Geometry: final body of the model. Coordinates: model frame, mm. Round coordinates to 2 decimals unless told otherwise and drop trailing zeros. Loops run counter-clockwise (first coordinate to the right, second up) from the corner with the lowest first, then second, coordinate; pieces in that order, holes last. Notation, with made-up numbers: M 9.25,-30.75 L 24.25,-30.75 A27 ccw 24.25,0.25 Z; hole C 74.25,1.5 d6. An arc over 180 degrees is marked long. Answer as a JSON object with one key per item and string values.
```python
from build123d import *

# Parameters (mm, degrees)
SKETCH1_R           = 2
SKETCH1_R_2         = 3
BOSS_EXTRUDE1_DEPTH = 5
SKETCH2_R           = 2
CUT_EXTRUDE1_DEPTH  = 36.174564674


with BuildPart() as part:
    # Sketch1 → Boss-Extrude1 (new body)
    with BuildSketch(Plane.XY):
        with BuildLine():
            Line((-3.972684511, 30.466666667), (-7.448783458, 0.875))
            ThreePointArc((-7.448783458, 0.875), (0, -7.5), (7.448783458, 0.875))
            Line((7.448783458, 0.875), (3.972684511, 30.466666667))
            ThreePointArc((3.972684511, 30.466666667), (0, 34), (-3.972684511, 30.466666667))
        make_face()
        with Locations((0, 30)):
            Circle(SKETCH1_R, mode=Mode.SUBTRACT)
        Circle(SKETCH1_R_2, mode=Mode.SUBTRACT)
    extrude(amount=BOSS_EXTRUDE1_DEPTH)

    # Sketch2 → Cut-Extrude1 (cut, through all)
    with BuildSketch(Plane.XY.offset(5)):
        with Locations((0, 15)):
            Circle(SKETCH2_R)
    extrude(amount=-CUT_EXTRUDE1_DEPTH, mode=Mode.SUBTRACT)


solid = part.part
```
1) Cut plane A-A on y = 0. Return the cut outline in (x, z).
Geometry results:
{"outline": "M -7.5,0 L -3,0 L -3,5 L -7.5,5 Z; M 3,0 L 7.5,0 L 7.5,5 L 3,5 Z"}
2) Pull-direction query (Y, two-part tool) for faces 1 (the face through (5.735, 15.464, 2.465)), 2 (the face through (-3, 0, 2)), 3 (the face through (2, 14, 5)), 4 (the face through (0, 17, 3)); classes: +Y half, -Y half, draft (parallel to the pull), parting line (faces both ways), or undercut.
Geometry results:
{"face 1": "+Y half", "face 2": "undercut", "face 3": "draft", "face 4": "undercut"}
3) First-contact query: pin 1 (3.5 mm diameter, centred on x = 0, y = 30, fed in from -Z); pin 2 (3 mm diameter, centred on x = -3, z = 3, fed in from -Y); pin 3 (2 mm diameter, centred on x = 3, z = 4.5, fed in from +Y). Flat tips, straight axial feed; report the tip coordinate or a pass-through.
Geometry results:
{"pin 1": "through", "pin 2": "y = -7.35", "pin 3": "y = 33.46"}
4) Cut plane B-B on x = 0. Return the cut outline in (y, z), and give its area (4 significant figures).
Geometry results:
{"outline": "M -7.5,0 L -3,0 L -3,5 L -7.5,5 Z; M 3,0 L 13,0 L 13,5 L 3,5 Z; M 17,0 L 28,0 L 28,5 L 17,5 Z; M 32,0 L 34,0 L 34,5 L 32,5 Z", "area": "137.5 mm2"}
5) Cut plane C-C on z = 1.8. Return the cut outline in (x, y) (3 decimals).
Geometry results:
{"outline": "M -7.449,0.875 A7.5 ccw long 7.449,0.875 L 3.973,30.467 A4 ccw -3.973,30.467 Z; hole C 0,0 d6; hole C 0,15 d4; hole C 0,30 d4"}
6) Cut plane D-D on y = 28.5. Return the cut outline in (x, z).
Geometry results:
{"outline": "M -4.2,0 L -1.32,0 L -1.32,5 L -4.2,5 Z; M 1.32,0 L 4.2,0 L 4.2,5 L 1.32,5 Z"}
7) Line query: probe 1 along Y at (x, z) = (0, 3.35); probe 2 along Y at (x, z) = (-1.5, 4.3); probe 3 along Y at (x, z) = (-2.75, 2.3). Output: solid intervals per line, ascending.
Geometry results:
{"probe 1": "-7.5 to -3, 3 to 13, 17 to 28, 32 to 34", "probe 2": "-7.35 to -2.6, 2.6 to 13.68, 16.32 to 28.68, 31.32 to 33.71", "probe 3": "-6.98 to -1.2, 1.2 to 32.9"}
